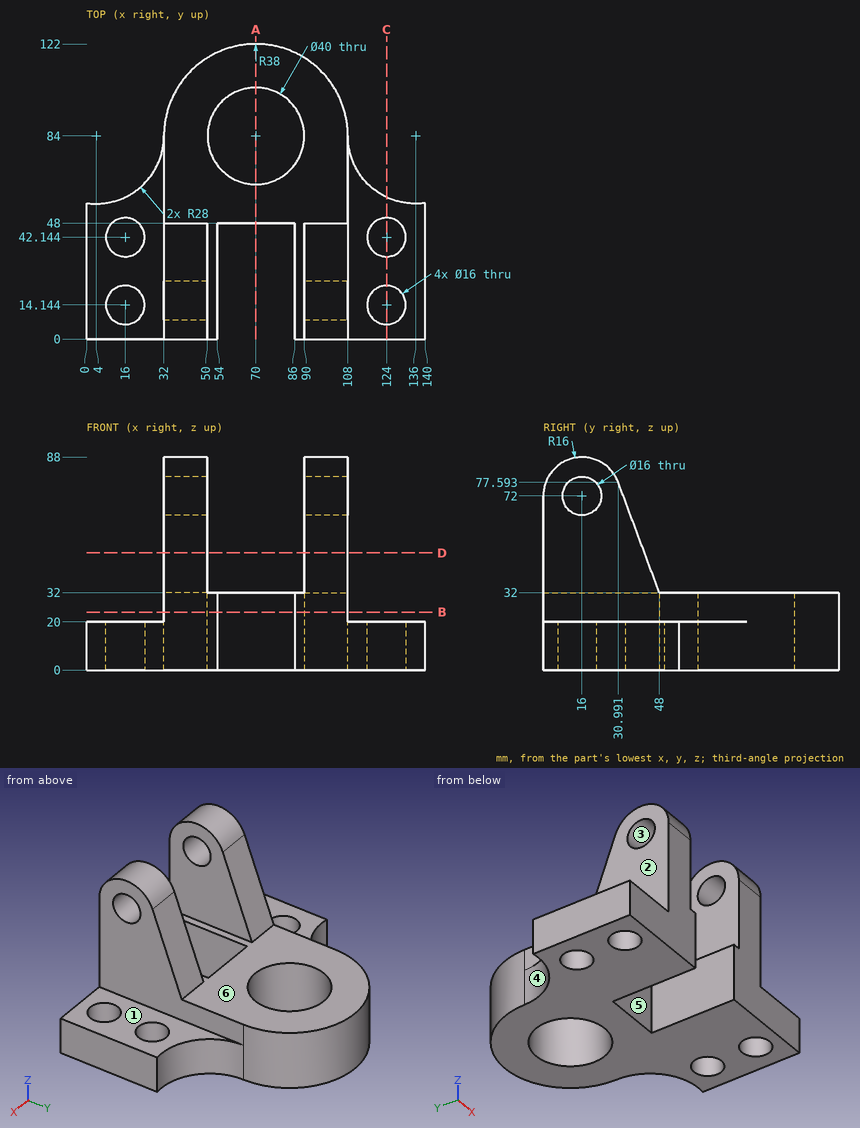
Verification items for this drawing (mm, ordinates from the low corner). A direction names the side the tool comes from. Coordinates: 2 decimals unless noted, no trailing zeros. Order: outer loops, then holes, each group sorted by start corner. A loop starts at its lowest first (then second) coordinate and runs counter-clockwise, first axis right, second up. Notation, with made-up numbers: (-10.5, 23.5) - (1.5, 23.5) arc R10 cw to (1.5, 40.5) - close; hole circle Ø5 at (77, 69.25). An arc over 180 degrees is marked (long way). Answer in a Markdown table with one row per item. Add a question column.
1. Gauge pin test, flat ends, axial feed: pin 1 Ø16 at (x, y) = (22.5, 25.5) entering from +Z; pin 2 Ø8 at (y, z) = (23, 45) entering from +X. Record the tip position at first contact, or that the pin passes through.
2. Material ranges on L1, parallel to X at y = 6, z = 30.5; L2, parallel to X at y = 33, z = 57; L3, parallel to Z at x = 42.25, y = 16, recorded low to high. Write a range as [from, to].
3. Draft check along Z on the marked faces 1, 2 and 3. Enter one of: +Z half, -Z half, draft (parallel to the pull), parting line (faces both ways), or undercut.
4. Section check A-A (x = 70). Enter the section's corners in (y, z), plus the area to 3 significant figures.
5. Section check D-D (z = 48.5). Enter the section's corners in (x, y) (1 decimal), plus the area to 3 significant figures.
6. Section check C-C (x = 124). Enter the section's corners in (y, z).
7. Access from +Z, -Z, +X, -X, +Y, -Y to the whole of each face (thin tool, end or side, straight path). Record for the marked faces 4, 5 and 6.
8. Section check B-B (z = 24). Enter the section's corners in (x, y).
Data:
| question | item | result |
|---|---|---|
| 1 | pin 1 | stops at z = 20 |
| 1 | pin 2 | stops at x = 108 |
| 2 | L1 | x = [32, 54], [86, 108] |
| 2 | L2 | x = [32, 50], [90, 108] |
| 2 | L3 | z = [0, 64], [80, 88] |
| 3 | face 1 | +Z half |
| 3 | face 2 | draft |
| 3 | face 3 | undercut |
| 4 | outline | (48, 0) - (64, 0) - (64, 32) - (48, 32) - close; (104, 0) - (122, 0) - (122, 32) - (104, 32) - close |
| 4 | area | 1,090 mm² |
| 5 | outline | (32, 0) - (50, 0) - (50, 41.8) - (32, 41.8) - close; (90, 0) - (108, 0) - (108, 41.8) - (90, 41.8) - close |
| 5 | area | 1,510 mm² |
| 6 | outline | (0, 0) - (6.14, 0) - (6.14, 20) - (0, 20) - close; (22.14, 0) - (34.14, 0) - (34.14, 20) - (22.14, 20) - close; (50.14, 0) - (58.7, 0) - (58.7, 20) - (50.14, 20) - close |
| 7 | face 4 | +Z, -Z, +Y |
| 7 | face 5 | +Z, -Z, -Y |
| 7 | face 6 | +Z, +Y |
| 8 | outline | (32, 0) - (54, 0) - (54, 48) - (86, 48) - (86, 0) - (108, 0) - (108, 84) arc R38 ccw to (32, 84) - close; hole circle Ø40 at (70, 84) |
